Read the model definition and answer for the solid it produces. Units are mm, in the model's axes. A direction names the side the tool comes from. Give positions to 0.01 mm unless a question says otherwise; leave off trailing zeros. Loops run counter-clockwise (first coordinate to the right, second up) from the corner with the lowest first, then second, coordinate; pieces in that order, holes last. Notation, with made-up numbers: (-6.5, 14.25) - (16.5, 14.25) arc R21 cw to (16.5, 25.25) - close; hole circle Ø2 at (62.5, -38.75). An arc over 180 degrees is marked (long way). Write each question's results on one line, items separated by ' | '. Start each with the question number.
Q1. The part is cut by section A-A, the plane x = 9. Write down the section's boundary in (y, z), plus the area to 3 significant figures.
Q2. The part is cut by section C-C, the plane z = 208. Write down the section's boundary in (x, y).
Q3. Determine the mould class of faces 1 (the flat face through (25, 0, 4)), 2 (the flat face through (-25, 0, 4)), 3 (the flat face through (0, 22, 4)), 4 (the flat face through (-22, 0, 4)) for opening direction X: +X half, -X half, draft (parallel to the pull), parting line (faces both ways), or undercut.
Q4. For faces 5 (the flat face through (0, -22, 4)), 6 (the flat face through (0, -25, 4)), determine the directions among +Z, -Z, +X, -X, +Y, -Y from which every point of the face is accessible in a straight line to the end or side of a thin tool.
Q5. Find the intervals of material crossed by line 1 (X direction, y = -2, z = 116); line 2 (Y direction, x = 23, z = -39.5), in increasing order. Write a range as from..to.
```python
from build123d import *

# Parameters (mm, degrees)
GB_6728_1986_050_X_50_X_3_1_DEPTH = 620


with BuildPart() as part:
    # Sketch1 → Gb／6728-1986方形空心型钢 050 X 50 X 3(1) (new body)
    with BuildSketch(Plane.YX.offset(-310)):
        with BuildLine():
            Line((-19, -25), (19, -25))
            ThreePointArc((19, -25), (23.242640687, -23.242640687), (25, -19))
            Line((25, -19), (25, 19))
            ThreePointArc((25, 19), (23.242640687, 23.242640687), (19, 25))
            Line((19, 25), (-19, 25))
            ThreePointArc((-19, 25), (-23.242640687, 23.242640687), (-25, 19))
            Line((-25, 19), (-25, -19))
            ThreePointArc((-25, -19), (-23.242640687, -23.242640687), (-19, -25))
        make_face()
        with BuildLine():
            Line((-19, -22), (19, -22))
            ThreePointArc((19, -22), (21.121320344, -21.121320344), (22, -19))
            Line((22, -19), (22, 19))
            ThreePointArc((22, 19), (21.121320344, 21.121320344), (19, 22))
            Line((19, 22), (-19, 22))
            ThreePointArc((-19, 22), (-21.121320344, 21.121320344), (-22, 19))
            Line((-22, 19), (-22, -19))
            ThreePointArc((-22, -19), (-21.121320344, -21.121320344), (-19, -22))
        make_face(mode=Mode.SUBTRACT)
    extrude(amount=GB_6728_1986_050_X_50_X_3_1_DEPTH)


solid = part.part
```
Check sheet entries:
1) outline: (-25, -310) - (-22, -310) - (-22, 310) - (-25, 310) - close; (22, -310) - (25, -310) - (25, 310) - (22, 310) - close | area: 3,720 mm^2
2) outline: (-25, -19) arc R6 ccw to (-19, -25) - (19, -25) arc R6 ccw to (25, -19) - (25, 19) arc R6 ccw to (19, 25) - (-19, 25) arc R6 ccw to (-25, 19) - close; hole (-22, -19) arc R3 ccw to (-19, -22) - (19, -22) arc R3 ccw to (22, -19) - (22, 19) arc R3 ccw to (19, 22) - (-19, 22) arc R3 ccw to (-22, 19) - close
3) face 1: +X half | face 2: -X half | face 3: undercut | face 4: undercut
4) face 5: +Z, -Z | face 6: +Z, -Z, +X, -X, -Y
5) line 1: x = -25..-22, 22..25 | line 2: y = -23.47..23.47
